Check sheet for the modelled part. Datum: model origin and axes. Units: mm. A direction names the side the tool comes from. Give positions to 0.01 mm unless a question says otherwise; leave off trailing zeros. Loops run counter-clockwise (first coordinate to the right, second up) from the corner with the lowest first, then second, coordinate; pieces in that order, holes last. Notation, with made-up numbers: M -32,89 L 26,89 A21 cw 26,119 Z; hole C 31.5,-26 d6. An arc over 180 degrees is marked long. Use one line per item in the form item = value.
from build123d import *

# Parameters (mm, degrees)
SKETCH_1_R           = 12.5
SKETCH_1_R_2         = 5
EXTRUDE_1_DEPTH      = 10
EXTRUDE_3_DEPTH      = 10
EXTRUDE_4_REACH      = 60.746
EXTRUDE_4_END_RADIUS = 12.5
SKETCH_6_W           = 20
SKETCH_6_H           = 20
HOLE_WIZARD_M6_1_D   = 5


with BuildPart() as part:
    # Sketch 1 → Extrude 1 (new, symmetric)
    with BuildSketch(Plane.XY):
        Circle(SKETCH_1_R)
        Circle(SKETCH_1_R_2, mode=Mode.SUBTRACT)
    extrude(amount=EXTRUDE_1_DEPTH, both=True)



with BuildPart() as body_2:
    # Sketch 5 → Extrude 3 (new, symmetric)
    with BuildSketch(Plane(origin=(0, 0, 0), x_dir=(0, 0, -1), z_dir=(1, 0, 0))):
        Polygon((10, -12.5), (21.657691454, -37.5), (41.168402769, -37.5), (41.168402769, -52.5), (-41.168402769, -52.5), (-41.168402769, -37.5), (-21.657691454, -37.5), (-10, -12.5), align=None)
    extrude(amount=EXTRUDE_3_DEPTH, both=True)


with BuildPart() as part_1:
    add(part.part)

    add(body_2.part)  # Extrude 4 merges body 2
    # Extrude 4: up to this cylinder (the profile starts outside it)
    extrude_4_end = Plane(origin=(0, 0, 0), z_dir=(0, 0, -1)) * Cylinder(EXTRUDE_4_END_RADIUS, 147.492, mode=Mode.PRIVATE)
    # Sketch 6 → Extrude 4 (add, up to the surface)
    with BuildSketch(Plane(origin=(0, -12.5, 0), x_dir=(1, 0, 0), z_dir=(0, 1, 0)), mode=Mode.PRIVATE) as extrude_4_sk1:
        Rectangle(SKETCH_6_W, SKETCH_6_H)
    extrude_4_tool1 = extrude(extrude_4_sk1.sketch, amount=EXTRUDE_4_REACH, mode=Mode.PRIVATE) - extrude_4_end
    add(extrude_4_tool1.solids().sort_by_distance((0, -12.5, 0))[0])
    add(extrude_4_tool1.solids().sort_by_distance((0, -12.5, 0))[1])

    # Hole Wizard M6 _1 (through all)
    with Locations(Plane(origin=(0, -37.5, -31.168402769), x_dir=(0, 0, 1), z_dir=(0, 1, 0))):
        with Locations((0, 0)):
            hole_wizard_m6_1 = Hole(HOLE_WIZARD_M6_1_D / 2)

    # Mirror 1: Hole Wizard M6 _1 across plane
    add(hole_wizard_m6_1.mirror(Plane.XY), mode=Mode.SUBTRACT)


solid = part_1.part
1) Release check for a two-part mould opening along X. For faces 4 (the face through (0.11, -45.1, 28.67)), 5 (the face through (0, -37.5, 34)), 6 (the face through (0.387, 12.494, 0.14)) record: pulls with the +X half, pulls with the -X half, needs draft (parallel to the pull), parting line crosses it, or undercut.
Evaluation:
face_4 = undercut
face_5 = needs draft
face_6 = parting line crosses it
2) Section check B-B (x = 0). Record the cut outline in (y, z), then the cut area to 3 significant figures.
Evaluation:
outline = M -52.5,-41.17 L -37.5,-41.17 L -37.5,-33.67 L -52.5,-33.67 Z; M -52.5,-28.67 L -37.5,-28.67 L -37.5,-21.66 L -12.5,-10 L -5,-10 L -5,10 L -12.5,10 L -37.5,21.66 L -37.5,28.67 L -52.5,28.67 Z; M -52.5,33.67 L -37.5,33.67 L -37.5,41.17 L -52.5,41.17 Z; M 5,-10 L 12.5,-10 L 12.5,10 L 5,10 Z
area = 2,180 mm^2
3) Set-up check for faces 1 (the face through (-2, -37.5, -29)), 2 (the face through (0, -6, 10)), 3 (the face through (-10, -35, 1)): record each of +Z, -Z, +X, -X, +Y, -Y from which the full face is reachable in a straight line by a thin tool's end or side.
Evaluation:
face_1 = -Z, +X, -X, +Y
face_2 = +Z, +X, -X, +Y
face_3 = +Z, -Z, -X, -Y
4) Scan lines: line 1 (X direction, y = -42, z = 27); line 2 (Y direction, x = 8, z = -31); line 3 (Y direction, x = -0.75, z = -1.5). Record each from-to range of solid material in increasing order.
Evaluation:
line_1 = -10 to 10
line_2 = -52.5 to -37.5
line_3 = -52.5 to -4.94, 4.94 to 12.48
5) Section check D-D (z = 36). Record the cut outline in (x, y).
Evaluation:
outline = M -10,-52.5 L 10,-52.5 L 10,-37.5 L -10,-37.5 Z
6) Depth check by flat-ended pin: pin 1 Ø1 at (y, z) = (-4, -7.5) entering from +X; pin 2 Ø2 at (x, y) = (9, 2) entering from +Z; pin 3 Ø3 at (x, y) = (9, -34) entering from +Z. Enter the tip coordinate at first touch or a pass-through.
Evaluation:
pin_1 = 12
pin_2 = 10
pin_3 = 20.73
7) Section check C-C (x = 6). Record the cut outline in (y, z).
Evaluation:
outline = M -52.5,-41.17 L -37.5,-41.17 L -37.5,-21.66 L -12.5,-10 L 10.97,-10 L 10.97,10 L -12.5,10 L -37.5,21.66 L -37.5,41.17 L -52.5,41.17 Z
8) Section check A-A (y = 0). Record the cut outline in (x, z), then the cut area to 3 significant figures.
Evaluation:
outline = M -12.5,-10 L -5,-10 L -5,10 L -12.5,10 Z; M 5,-10 L 12.5,-10 L 12.5,10 L 5,10 Z
area = 300 mm^2
